```python
from build123d import *

# Parameters (mm, degrees)
SKETCH_1_W                   = 170
SKETCH_1_H                   = 14
EXTRUDE_1_DEPTH              = 5
HOLE_WIZARD_M6_1_D           = 5
HOLE_WIZARD_M6_1_CSINK_D     = 6.05
HOLE_WIZARD_M6_1_CSINK_ANGLE = 90


with BuildPart() as part:
    # 草图1 → 凸台-拉伸1 (new, symmetric)
    with BuildSketch(Plane.XY):
        Rectangle(SKETCH_1_W, SKETCH_1_H)
    extrude(amount=EXTRUDE_1_DEPTH, both=True)

    # M6 螺纹孔1 (through all)
    with Locations(Plane(origin=(-73, 0, -5), x_dir=(-1, 0, 0), z_dir=(0, 0, -1))):
        with Locations((0, 0)):
            hole_wizard_m6_1 = CounterSinkHole(HOLE_WIZARD_M6_1_D / 2, HOLE_WIZARD_M6_1_CSINK_D / 2, counter_sink_angle=HOLE_WIZARD_M6_1_CSINK_ANGLE)

    # 镜向1: M6 螺纹孔1 across plane
    add(hole_wizard_m6_1.mirror(Plane(origin=(0, 0, 0), x_dir=(0, 0, 1), z_dir=(1, 0, 0))), mode=Mode.SUBTRACT)


solid = part.part
```
Could you check a few things on this model? Use its own coordinates, in mm. Round coordinates to 2 decimals unless told otherwise and drop trailing zeros. Loops run counter-clockwise (first coordinate to the right, second up) from the corner with the lowest first, then second, coordinate; pieces in that order, holes last. Notation, with made-up numbers: M -21.5,34 L -7.5,34 A25 ccw -7.5,68 Z; hole C 58,49 d7. An arc over 180 degrees is marked long. Write item = value, one per line.
1. I want a section at A-A, the plane x = 73. Write out the boundary of the cut face in (y, z) (3 decimals).
Results below:
outline = M -7,-5 L -3.025,-5 L -2.5,-4.475 L -2.5,5 L -7,5 Z; M 2.5,-4.475 L 3.025,-5 L 7,-5 L 7,5 L 2.5,5 Z
2. Will this pin go through, and if not, where does the flat tip stop? P1, Ø4, axis at x = 73, y = 0, coming from the -Z side.
Results below:
P1 = through
3. Thinking about a two-plate mould opening in Y: for faces 1 (the face through (-1, -7, 0)), 2 (the face through (-85, 0, 0)), 3 (the face through (-1, 7, 0)), 4 (the face through (-75.5, 0.1, 0.3)), which applies, +Y half, -Y half, draft (parallel to the pull), parting line (faces both ways), or undercut?
Results below:
face_1 = -Y half
face_2 = draft
face_3 = +Y half
face_4 = undercut
4. I want a section at C-C, the plane y = 0. Write out the boundary of the cut face in (x, z) (3 decimals).
Results below:
outline = M -85,-5 L -76.025,-5 L -75.5,-4.475 L -75.5,5 L -85,5 Z; M -70.5,-4.475 L -69.975,-5 L 69.975,-5 L 70.5,-4.475 L 70.5,5 L -70.5,5 Z; M 75.5,-4.475 L 76.025,-5 L 85,-5 L 85,5 L 75.5,5 Z
5. I want a section at B-B, the plane z = -1.25. Write out the boundary of the cut face in (x, y), and give its area (3 significant figures).
Results below:
outline = M -85,-7 L 85,-7 L 85,7 L -85,7 Z; hole C -73,0 d5; hole C 73,0 d5
area = 2,340 mm²
6. I need wall thicknesses on probe 1 along X at (y, z) = (0, 3.25); probe 2 along Y at (x, z) = (-73, -2); probe 3 along X at (y, z) = (-0.5, -1.5). Which ranges of each line are inside material? Lowest first, please.
Results below:
probe_1 = -85 to -75.5, -70.5 to 70.5, 75.5 to 85
probe_2 = -7 to -2.5, 2.5 to 7
probe_3 = -85 to -75.45, -70.55 to 70.55, 75.45 to 85
